```python
from build123d import *

# Parameters (mm, degrees)
BASE_PLATE_DEPTH                      = 100
V_BLOCK_UPRIGHTS_DEPTH                = 25
M6_TAPPED_HOLES_2X_D                  = 5
M6_TAPPED_HOLES_2X_DEPTH              = 18.497848452
M6_TAPPED_HOLES_2X_CSINK_D            = 6.05
M6_TAPPED_HOLES_2X_CSINK_ANGLE        = 90
M6_TAPPED_HOLES_2X_TIP                = 1.502151548
CENTRE_STEP_BLOCK_PROFILE_R           = 5
CENTRE_STEP_BLOCK_DEPTH               = 12
ADJUSTMENT_SLOT_AND_CENTRE_HOLE_DEPTH = 108.930533215


with BuildPart() as part:
    # Base Plate Profile → Base Plate (new body)
    with BuildSketch(Plane.XY):
        Polygon((25, 0), (-25, 0), (-25, -6), (-32, -6), (-32, 13), (32, 13), (32, -6), (25, -6), align=None)
    extrude(amount=-BASE_PLATE_DEPTH)

    # V-Block Uprights Profile → V-Block Uprights (add)
    with BuildSketch(Plane(origin=(0, 13, 0), x_dir=(1, 0, 0), z_dir=(0, 1, 0))):
        Polygon((32, 100), (32, 62), (19, 62), (12, 100), align=None)
        Polygon((-12, 100), (-32, 100), (-32, 62), (-19, 62), align=None)
    extrude(amount=V_BLOCK_UPRIGHTS_DEPTH)

    # M6 Tapped Holes 2x
    with Locations(Plane(origin=(0, 38, 0), x_dir=(1, 0, 0), z_dir=(0, 1, 0))):
        with Locations((22, 87), (-22, 87)):
            CounterSinkHole(M6_TAPPED_HOLES_2X_D / 2, M6_TAPPED_HOLES_2X_CSINK_D / 2, depth=M6_TAPPED_HOLES_2X_DEPTH, counter_sink_angle=M6_TAPPED_HOLES_2X_CSINK_ANGLE)
            with Locations((0, 0, -(M6_TAPPED_HOLES_2X_DEPTH + M6_TAPPED_HOLES_2X_TIP / 2))):  # 118° drill point
                Cone(0, M6_TAPPED_HOLES_2X_D / 2, M6_TAPPED_HOLES_2X_TIP, mode=Mode.SUBTRACT)

    # Centre Step Block Profile → Centre Step Block (add)
    with BuildSketch(Plane(origin=(0, 13, 0), x_dir=(1, 0, 0), z_dir=(0, 1, 0))):
        Polygon((-12, 100), (12, 100), (19, 62), (-19, 62), align=None)
        with Locations(Location((0, 81, 0), (0, 0, 180))):
            Circle(CENTRE_STEP_BLOCK_PROFILE_R, mode=Mode.SUBTRACT)
    extrude(amount=CENTRE_STEP_BLOCK_DEPTH)

    # Adjustment Slot and Centre Hole Profile → Adjustment Slot and Centre Hole (cut, through all)
    with BuildSketch(Plane(origin=(0, 13, 0), x_dir=(1, 0, 0), z_dir=(0, 1, 0))):
        with BuildLine():
            Line((-9, 20), (-9, 40))
            ThreePointArc((-9, 40), (0, 49), (9, 40))
            Line((9, 40), (9, 20))
            ThreePointArc((9, 20), (0, 11), (-9, 20))
        make_face()
    extrude(amount=-ADJUSTMENT_SLOT_AND_CENTRE_HOLE_DEPTH, mode=Mode.SUBTRACT)


solid = part.part
```
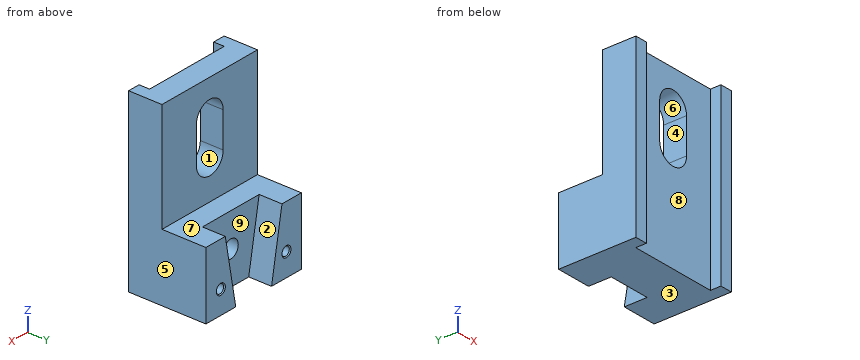
Geometry check sheet. Reference: the model listing, model coordinates, mm. Face numbers are marked on the shaded views. A direction names the side the tool comes from. Give positions to 0.01 mm unless a question says otherwise; leave off trailing zeros. Loops run counter-clockwise (first coordinate to the right, second up) from the corner with the lowest first, then second, coordinate; pieces in that order, holes last. Notation, with made-up numbers: (-8.5, 67.5) - (17.5, 67.5) arc R23 ccw to (17.5, 82.5) - close; hole circle Ø2 at (83.5, -30.5). An arc over 180 degrees is marked (long way). Use CSV: the item, a comma, the result in double quotes. Start each with the question number.
Q1. Section check C-C, the plane y = -3. Record the cut outline in (x, z), and give its area (3 significant figures).
Q2. Section check D-D, the plane y = 6. Record the cut outline in (x, z).
Q3. Go/stop test with flat-tipped pins: pin 1 Ø4 at (x, z) = (22, -87) entering from -Y; pin 2 Ø6 at (x, z) = (1, -75.5) entering from +Y; pin 3 Ø4 at (x, z) = (14, -25.5) entering from +Y. Record where each tip stops, or that it passes through.
Q4. Access from +Z, -Z, +X, -X, +Y, -Y to the whole of each face (thin tool, end or side, straight path). Record for the marked faces 5, 6, 7, 8 and 9.
Q5. Scan lines: probe 1 along Z at (x, y) = (22, 29); probe 2 along Z at (x, y) = (0, 22.75); probe 3 along X at (y, z) = (28, -87). Record each from-to range of solid material in increasing order. Write a range as from..to.
Q6. Section check A-A, the plane x = 0. Record the cut outline in (y, z).
Q7. Section check B-B, the plane z = -34. Record the cut outline in (x, y), and give its area (3 significant figures).
Q8. Release check for a two-part mould opening along Z. For the marked faces 1, 2, 3 and 4 record: +Z half, -Z half, draft (parallel to the pull), parting line (faces both ways), or undercut.
Findings below:
1,outline,"(-32, -100) - (-25, -100) - (-25, 0) - (-32, 0) - close; (25, -100) - (32, -100) - (32, 0) - (25, 0) - close"
1,area,"1,400 mm^2"
2,outline,"(-32, -100) - (32, -100) - (32, 0) - (-32, 0) - close; hole (-9, -40) arc R9 ccw to (9, -40) - (9, -20) arc R9 ccw to (-9, -20) - close"
3,pin 1,"stops at y = 0"
3,pin 2,"stops at y = 25"
3,pin 3,"stops at y = 13"
4,face 5,"+Z, -Z, +X, +Y, -Y"
4,face 6,"+Y, -Y"
4,face 7,"+Z, +X, -X, +Y"
4,face 8,"+Z, -Z, -Y"
4,face 9,"+Z, +Y"
5,probe 1,"z = -100..-89.5, -84.5..-62"
5,probe 2,"z = -100..-86, -76..-62"
5,probe 3,"x = -32..-24.5, -19.5..-14.39, 14.39..19.5, 24.5..32"
6,outline,"(0, -100) - (25, -100) - (25, -86) - (13, -86) - (13, -76) - (25, -76) - (25, -62) - (13, -62) - (13, -49) - (0, -49) - close; (0, -11) - (13, -11) - (13, 0) - (0, 0) - close"
7,outline,"(-32, -6) - (-25, -6) - (-25, 0) - (-9, 0) - (-9, 13) - (-32, 13) - close; (9, 0) - (25, 0) - (25, -6) - (32, -6) - (32, 13) - (9, 13) - close"
7,area,"682 mm^2"
8,face 1,"undercut"
8,face 2,"+Z half"
8,face 3,"-Z half"
8,face 4,"undercut"
